Source: three-view drawing plus pictorial views. Frame: mm from the lowest corner of the part. Round coordinates to 2 decimals unless told otherwise and drop trailing zeros. Order: outer loops, then holes, each group sorted by start corner. A loop starts at its lowest first (then second) coordinate and runs counter-clockwise, first axis right, second up. Notation, with made-up numbers: (29.25, 0.25) -> (68.25, 0.25) arc R30 cw to (68.25, 23.25) -> close; hole circle Ø2 at (-27.5, -15.5). An arc over 180 degrees is marked (long way). Use a Markdown table: item, result.
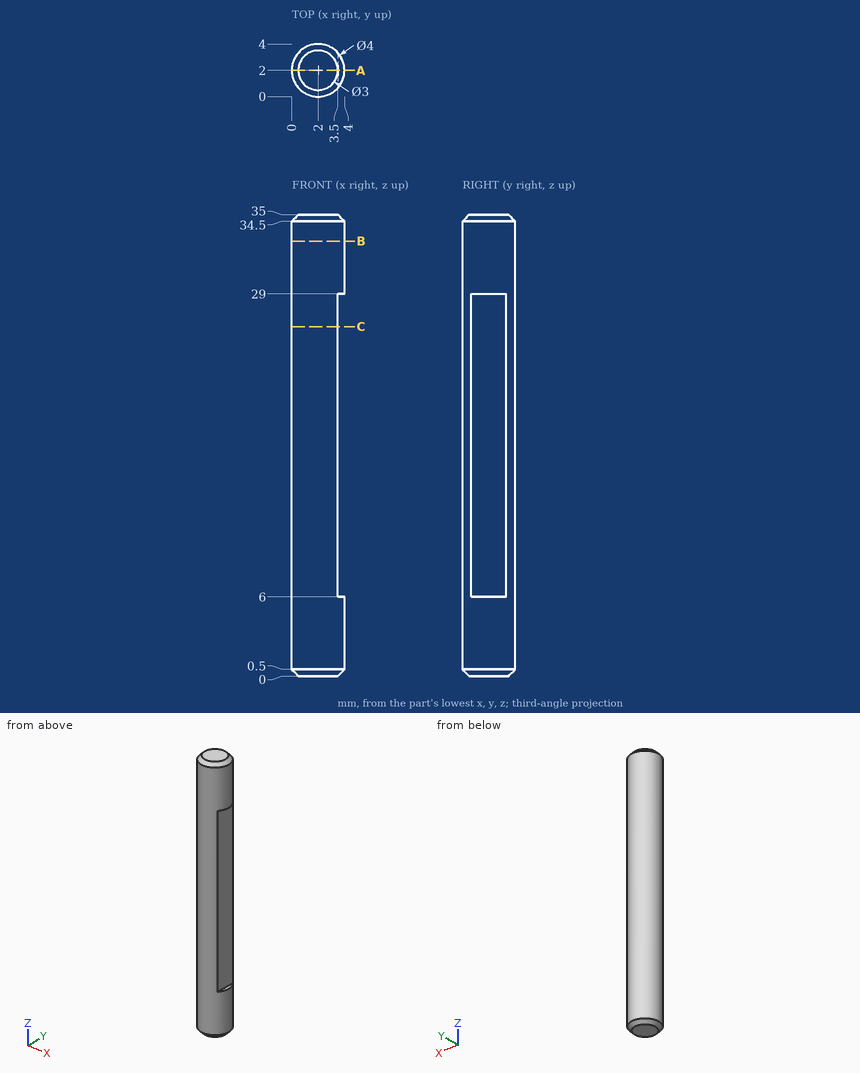
1) Cut plane C-C on z = 26.5. Return loops of the section in (x, y).
Results found:
| item | result |
|---|---|
| outline | (3.5, 0.68) -> (3.5, 3.32) arc R2 ccw (long way) to start |
2) Cut plane B-B on z = 33. Return loops of the section in (x, y).
Results found:
| item | result |
|---|---|
| outline | circle Ø4 at (2, 2) |
3) Line query: L1, parallel to X at y = 2.15, z = 10; L2, parallel to Y at x = 2.1, z = 22; L3, parallel to Y at x = 1.2, z = 2.5. Output: solid intervals per line, ascending. Write a range as [from, to].
Results found:
| item | result |
|---|---|
| L1 | x = [0.01, 3.5] |
| L2 | y = [0, 4] |
| L3 | y = [0.17, 3.83] |
4) Pin query (flat end, axial travel): pin 1 Ø1 at (x, z) = (3.5, 29) entering from -Y; pin 2 Ø1.3 at (y, z) = (2.5, 15) entering from +X; pin 3 Ø0.6 at (x, y) = (3.5, 1.5) entering from +Z. Return the tip coordinate at first contact, or that it passes through.
Results found:
| item | result |
|---|---|
| pin 1 | stops at y = 0.27 |
| pin 2 | stops at x = 3.5 |
| pin 3 | stops at z = 35 |
5) Cut plane A-A on y = 2. Return loops of the section in (x, z), and give its area (3 significant figures).
Results found:
| item | result |
|---|---|
| outline | (0, 0.5) -> (0.5, 0) -> (3.5, 0) -> (4, 0.5) -> (4, 6) -> (3.5, 6) -> (3.5, 29) -> (4, 29) -> (4, 34.5) -> (3.5, 35) -> (0.5, 35) -> (0, 34.5) -> close |
| area | 128 mm² |
